Geometry: final body of the model. Coordinates: model frame, mm. A direction names the side the tool comes from. Give positions to 0.01 mm unless a question says otherwise; leave off trailing zeros. Loops run counter-clockwise (first coordinate to the right, second up) from the corner with the lowest first, then second, coordinate; pieces in that order, holes last.
1. Material intervals for line 1 along Y through (x, z) = (0, 3.75); line 2 along Y through (x, z) = (0, -12.25); line 3 along Y through (x, z) = (0.5, -788), sorted ascending.
2. Access query for faces 1 (the face through (-17, -6, -170)), 2 (the face through (8.06, -12.65, -1370.24)), 3 (the face through (-3, -13, -1350)), 4 (the face through (3, -3, 10)). Directions: +Z, -Z, +X, -X, +Y, -Y. A direction counts if a zero-diameter tool reaches every point of the face in a straight line with its end or side. Return the directions, or none.
3. Section B-B, the plane z = -998. Output: boundary loops of the cut face in (x, y).
4. Section A-A, the plane z = -120. Output: boundary loops of the cut face in (x, y), then the cut area to 3 significant figures.
5. First-contact query: P1, Ø1.5, axis at y = -10, z = -993.5, coming from the +X side; P2, Ø1.5, axis at y = 15.5, z = -410, coming from the +X side; P3, Ø3, axis at y = 12.5, z = -43, coming from the +X side. Flat tips, straight axial feed; report the tip coordinate or a pass-through.
6. Draft query along Z for faces 5 (the face through (-3.794, 17.084, -127.412)), 6 (the face through (10.316, -7.91, -1350.986)), 7 (the face through (-17, -6, -1270)), 8 (the face through (-0.1, -13.4, -1352)). Return one class per face: +Z half, -Z half, draft (parallel to the pull), parting line (faces both ways), or undercut.
from build123d import *

# Parameters (mm, degrees)
SKETCH_2_R             = 15
EXTRUDE_1_DEPTH        = 96
SKETCH_3_R             = 17.5
EXTRUDE_2_DEPTH        = 84
SKETCH_4_R             = 20
EXTRUDE_3_DEPTH        = 1100
SKETCH_6_R             = 17.5
EXTRUDE_4_DEPTH        = 80
SKETCH_7_R             = 13
EXTRUDE_5_DEPTH        = 2
SKETCH_9_R             = 15
EXTRUDE_6_DEPTH        = 38
CHAMFER_1_SIZE         = 1
CHAMFER_2_SIZE         = 1
CHAMFER_3_SIZE         = 1
CHAMFER_4_SIZE         = 1
HOLE_WIZARD_M8_2_D     = 6.8
HOLE_WIZARD_M8_2_DEPTH = 28.75
HOLE_WIZARD_M8_2_TIP   = 2.042926105
CUT_EXTRUDE_1_DEPTH    = 1391.489482161


with BuildPart() as part:
    # 草图2 → 凸台-拉伸1 (new body)
    with BuildSketch(Plane.XY):
        Circle(SKETCH_2_R)
    extrude(amount=-EXTRUDE_1_DEPTH)

    # 草图3 → 凸台-拉伸2 (add)
    with BuildSketch(Plane(origin=(0, 0, -96), x_dir=(-1, 0, 0), z_dir=(0, 0, -1))):
        with Locations(Location((0, 0, 0), (0, 0, 180))):
            Circle(SKETCH_3_R)
    extrude(amount=EXTRUDE_2_DEPTH)

    # 草图4 → 凸台-拉伸3 (add)
    with BuildSketch(Plane(origin=(0, 0, -180), x_dir=(-1, 0, 0), z_dir=(0, 0, -1))):
        Circle(SKETCH_4_R)
    extrude(amount=EXTRUDE_3_DEPTH)

    # 草图6 → 凸台-拉伸4 (add)
    with BuildSketch(Plane(origin=(0, 0, -1280), x_dir=(-1, 0, 0), z_dir=(0, 0, -1))):
        with Locations(Location((0, 0, 0), (0, 0, 180))):
            Circle(SKETCH_6_R)
    extrude(amount=EXTRUDE_4_DEPTH)

    # 草图7 → 凸台-拉伸5 (add)
    with BuildSketch(Plane(origin=(0, 0, -1360), x_dir=(-1, 0, 0), z_dir=(0, 0, -1))):
        Circle(SKETCH_7_R)
    extrude(amount=EXTRUDE_5_DEPTH)

    # 草图9 → 凸台-拉伸6 (add)
    with BuildSketch(Plane(origin=(0, 0, -1362), x_dir=(-1, 0, 0), z_dir=(0, 0, -1))):
        with Locations(Location((0, 0, 0), (0, 0, 180))):
            Circle(SKETCH_9_R)
    extrude(amount=EXTRUDE_6_DEPTH)

    # 倒角1
    chamfer_1_edges = [part.edges().sort_by_distance(p)[0] for p in [
        (-15, 0, -1400),
    ]]
    chamfer(chamfer_1_edges, length=CHAMFER_1_SIZE)

    # 倒角2
    chamfer_2_edges = [part.edges().sort_by_distance(p)[0] for p in [
        (20, 0, -1280),
    ]]
    chamfer(chamfer_2_edges, length=CHAMFER_2_SIZE)

    # 倒角3
    chamfer_3_edges = [part.edges().sort_by_distance(p)[0] for p in [
        (20, 0, -180),
    ]]
    chamfer(chamfer_3_edges, length=CHAMFER_3_SIZE)

    # 倒角4
    chamfer_4_edges = [part.edges().sort_by_distance(p)[0] for p in [
        (-15, 0, 0),
    ]]
    chamfer(chamfer_4_edges, length=CHAMFER_4_SIZE)


with BuildPart() as part_1:
    # Move Body 1: moved
    add(part.part.moved(Location((0, 0, 10))))

    # M8 螺纹孔2
    with Locations(Plane.XY.offset(10)):
        with Locations((0, 0)):
            Hole(HOLE_WIZARD_M8_2_D / 2, depth=HOLE_WIZARD_M8_2_DEPTH)
            with Locations((0, 0, -(HOLE_WIZARD_M8_2_DEPTH + HOLE_WIZARD_M8_2_TIP / 2))):  # 118° drill point
                Cone(0, HOLE_WIZARD_M8_2_D / 2, HOLE_WIZARD_M8_2_TIP, mode=Mode.SUBTRACT)

    # 草图18 → 切除-拉伸1 (cut, through all)
    with BuildSketch(Plane(origin=(0, 11, 0), x_dir=(1, 0, 0), z_dir=(0, 1, 0))):
        with BuildLine():
            Line((4, 77), (4, 5))
            ThreePointArc((4, 5), (0, 1), (-4, 5))
            Line((-4, 5), (-4, 77))
            ThreePointArc((-4, 77), (0, 81), (4, 77))
        make_face()
    extrude(amount=CUT_EXTRUDE_1_DEPTH, mode=Mode.SUBTRACT)


solid = part_1.part
Answers below:
1. line 1: y = -15 to -3.4, 3.4 to 15
1. line 2: y = -15 to -3.4, 3.4 to 11
1. line 3: y = -19.99 to 19.99
2. face 1: +Z
2. face 2: -Z
2. face 3: none
2. face 4: +Z, +X, -X, +Y, -Y
3. outline: circle Ø40 at (0, 0)
4. outline: circle Ø35 at (0, 0)
4. area: 962 mm2
5. P1: stops at x = 17.73
5. P2: stops at x = 13.51
5. P3: stops at x = 10.2
6. face 5: draft
6. face 6: undercut
6. face 7: -Z half
6. face 8: undercut
